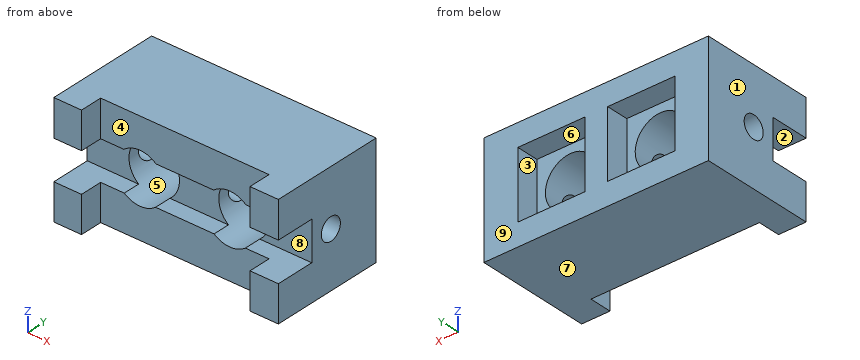
```python
from build123d import *

# Parameters (mm, degrees)
BASE_BLOCK_40_DEPTH          = 40
SQUARE_POCKETS_SKETCH_W      = 24
SQUARE_POCKETS_SKETCH_H      = 24
SQUARE_POCKETS_2X24X24_DEPTH = 8
POCKET_HOLES_SKETCH_R        = 9
POCKET_HOLES_2X_12_DEPTH     = 66.566879024
END_BORE_AND_SLOT_SKETCH_R   = 4
END_BORE_AND_SLOT_SKETCH_W   = 14
END_BORE_AND_SLOT_SKETCH_H   = 14
END_BORE_AND_SLOT_DEPTH      = 96.336247042


with BuildPart() as part:
    # Block Profile Sketch → Base Block 40 (new body)
    with BuildSketch(Plane.XY):
        Polygon((-30, 0), (30, 0), (30, -8), (40.125, -8), (40.125, 33), (-39.875, 33), (-39.875, -8), (-30, -8), align=None)
    extrude(amount=-BASE_BLOCK_40_DEPTH)

    # Square Pockets Sketch → Square Pockets 2x24x24 (cut)
    with BuildSketch(Plane(origin=(0, 33, 0), x_dir=(1, 0, 0), z_dir=(0, 1, 0))):
        with Locations((-16, 20)):
            Rectangle(SQUARE_POCKETS_SKETCH_W, SQUARE_POCKETS_SKETCH_H)
        with Locations((16, 20)):
            Rectangle(SQUARE_POCKETS_SKETCH_W, SQUARE_POCKETS_SKETCH_H)
    extrude(amount=-SQUARE_POCKETS_2X24X24_DEPTH, mode=Mode.SUBTRACT)

    # Pocket Holes Sketch → Pocket Holes 2xØ12 (cut, through all)
    with BuildSketch(Plane(origin=(0, 25, 0), x_dir=(1, 0, 0), z_dir=(0, 1, 0))):
        with Locations(Location((-16, 20, 0), (0, 0, 270))):
            Circle(POCKET_HOLES_SKETCH_R)
        with Locations(Location((16, 20, 0), (0, 0, 90))):
            Circle(POCKET_HOLES_SKETCH_R)
    extrude(amount=-POCKET_HOLES_2X_12_DEPTH, mode=Mode.SUBTRACT)

    # End Bore and Slot Sketch → End Bore and Slot (cut, through all)
    with BuildSketch(Plane(origin=(40.125, 0, 0), x_dir=(0, 0, -1), z_dir=(1, 0, 0))):
        with Locations(Location((20.067495301, 14, 0), (0, 0, 90))):
            Circle(END_BORE_AND_SLOT_SKETCH_R)
        with Locations((20.067495301, -1)):
            Rectangle(END_BORE_AND_SLOT_SKETCH_W, END_BORE_AND_SLOT_SKETCH_H)
    extrude(amount=-END_BORE_AND_SLOT_DEPTH, mode=Mode.SUBTRACT)


solid = part.part
```
Check sheet for the modelled part. Datum: model origin and axes. Units: mm. Face numbers are marked on the shaded views. A direction names the side the tool comes from. Coordinates: 2 decimals unless noted, no trailing zeros. Write each loop counter-clockwise with the first axis right and the second up, starting at its lowest first coordinate (ties: lowest second). Pieces come first, ordered by that corner, then holes. Notation, with made-up numbers: M -18.5,87 L 30.5,87 A31 ccw 30.5,116 Z; hole C -3,-22.75 d3. An arc over 180 degrees is marked long. Use one line per item in the form item = value.
Item 1: Sectioned sample at D-D, the plane z = -22. State how many separate pieces and enclosed holes the cut face has, and give its area (3 significant figures).
Answer below:
separate_pieces = 6
enclosed_holes = 0
area = 795 mm^2
Item 2: Release check for a two-part mould opening along Z. For the marked faces 6, 7, 8 and 9 record: pulls with the +Z half, pulls with the -Z half, needs draft (parallel to the pull), parting line crosses it, or undercut.
Answer below:
face_6 = undercut
face_7 = pulls with the -Z half
face_8 = undercut
face_9 = needs draft
Item 3: Sectioned sample at B-B, the plane y = 19.5. Record the cut outline in (x, z) (3 decimals).
Answer below:
outline = M -39.875,-40 L 40.125,-40 L 40.125,0 L -39.875,0 Z; hole C -16,-20 d18; hole C 16,-20 d18
Item 4: Set-up check for the marked faces 1, 2, 3, 4 and 5: record each of +Z, -Z, +X, -X, +Y, -Y from which the full face is reachable in a straight line by a thin tool's end or side.
Answer below:
face_1 = +Z, -Z, -X, +Y, -Y
face_2 = +X, -X, -Y
face_3 = +Y
face_4 = +Z, -Z, -Y
face_5 = +Y, -Y
Item 5: Sectioned sample at C-C, the plane y = 4.5. Record the cut outline in (x, z) (1 decimal), and give its area (3 significant figures).
Answer below:
outline = M -39.9,-40 L 40.1,-40 L 40.1,-27.1 L 21.6,-27.1 A9 cw 10.4,-27.1 L -10.4,-27.1 A9 cw -21.6,-27.1 L -39.9,-27.1 Z; M -39.9,-13.1 L -21.7,-13.1 A9 cw -10.3,-13.1 L 10.3,-13.1 A9 cw 21.7,-13.1 L 40.1,-13.1 L 40.1,0 L -39.9,0 Z
area = 2,020 mm^2
Item 6: Gauge pin test, flat ends, axial feed: pin 1 Ø2 at (x, z) = (16, -36) entering from -Y; pin 2 Ø15.5 at (x, y) = (-34, -3.5) entering from +Z; pin 3 Ø2 at (x, z) = (-25.5, -21) entering from -Y. Record the tip position at first contact, or that the pin passes through.
Answer below:
pin_1 = 0
pin_2 = 0
pin_3 = 6
Item 7: Material ranges on L1, parallel to Z at x = 33.5, y = 14; L2, parallel to X at y = 8, z = -20 (3 decimals); L3, parallel to X at y = 10.5, z = -18 (3 decimals), recorded low to high. Write a range as from..to.
Answer below:
L1 = -40..-24.07, -16.07..0
L2 = -39.875..-25, -7..7, 25..40.125
L3 = -39.875..-24.775, -7.225..7.225, 24.775..40.125
Item 8: Sectioned sample at A-A, the plane x = -16. Record the cut outline in (y, z), and give its area (3 significant figures).
Answer below:
outline = M 0,-40 L 33,-40 L 33,-32 L 25,-32 L 25,-29 L 0,-29 Z; M 0,-11 L 25,-11 L 25,-8 L 33,-8 L 33,0 L 0,0 Z
area = 678 mm^2
